from build123d import *

# Parameters (mm, degrees)
SKETCH1_W             = 70
SKETCH1_H             = 40
BOSS_EXTRUDE1_DEPTH   = 15
SKETCH2_W             = 60
SKETCH2_H             = 30
CUT_EXTRUDE1_DEPTH    = 51.249378106
CHAMFER1_SIZE         = 0.5
M4_TAPPED_HOLE1_D     = 3.3
M4_TAPPED_HOLE1_DEPTH = 11.5
M4_TAPPED_HOLE1_TIP   = 0.991420021
M4_TAPPED_HOLE2_D     = 3.3
CHAMFER3_SIZE         = 3
SKETCH17_W            = 10
SKETCH17_H            = 30
BOSS_EXTRUDE2_DEPTH   = 68.5
CHAMFER4_SIZE         = 0.5
M4_TAPPED_HOLE3_D     = 3.3
M4_TAPPED_HOLE3_DEPTH = 11.5
M4_TAPPED_HOLE3_TIP   = 0.991420021
CHAMFER5_SIZE         = 2
SKETCH20_R            = 2.5
CUT_EXTRUDE2_DEPTH    = 8
SKETCH21_W            = 3
SKETCH21_H            = 30
CUT_EXTRUDE3_DEPTH    = 114.829916981
CHAMFER6_SIZE         = 2


with BuildPart() as part:
    # Sketch1 → Boss-Extrude1 (new, symmetric)
    with BuildSketch(Plane.XY):
        Rectangle(SKETCH1_W, SKETCH1_H)
    extrude(amount=BOSS_EXTRUDE1_DEPTH, both=True)

    # Sketch2 → Cut-Extrude1 (cut, through all)
    with BuildSketch(Plane.XY.offset(15)):
        with Locations((-5, -5)):
            Rectangle(SKETCH2_W, SKETCH2_H)
    extrude(amount=-CUT_EXTRUDE1_DEPTH, mode=Mode.SUBTRACT)

    # Chamfer1
    chamfer1_edges = [part.edges().sort_by_distance(p)[0] for p in [
        (35, 0, 15),
        (35, 0, -15),
    ]]
    chamfer(chamfer1_edges, length=CHAMFER1_SIZE)

    # M4 Tapped Hole1
    with Locations(Plane(origin=(0, 20, 0), x_dir=(1, 0, 0), z_dir=(0, 1, 0))):
        with Locations((11, 0), (26, 0)):
            Hole(M4_TAPPED_HOLE1_D / 2, depth=M4_TAPPED_HOLE1_DEPTH)
            with Locations((0, 0, -(M4_TAPPED_HOLE1_DEPTH + M4_TAPPED_HOLE1_TIP / 2))):  # 118° drill point
                Cone(0, M4_TAPPED_HOLE1_D / 2, M4_TAPPED_HOLE1_TIP, mode=Mode.SUBTRACT)

    # M4 Tapped Hole2 (through all)
    with Locations(Plane(origin=(35, 0, 0), x_dir=(0, 0, -1), z_dir=(1, 0, 0))):
        with Locations((-10, 5), (-10, -15), (10, -15), (10, 5)):
            Hole(M4_TAPPED_HOLE2_D / 2)

    # Chamfer3
    chamfer3_edges = [part.edges().sort_by_distance(p)[0] for p in [
        (29.75, -20, -15),
        (29.75, -20, 15),
    ]]
    chamfer(chamfer3_edges, length=CHAMFER3_SIZE)

    # Sketch17 → Boss-Extrude2 (add)
    with BuildSketch(Plane(origin=(0, 20, 0), x_dir=(1, 0, 0), z_dir=(0, 1, 0))):
        with Locations((-30, 0)):
            Rectangle(SKETCH17_W, SKETCH17_H)
    extrude(amount=BOSS_EXTRUDE2_DEPTH)

    # Chamfer4
    chamfer4_edges = [part.edges().sort_by_distance(p)[0] for p in [
        (-25, 88.5, 0),
        (-35, 88.5, 0),
    ]]
    chamfer(chamfer4_edges, length=CHAMFER4_SIZE)

    # M4 Tapped Hole3
    with Locations(Plane(origin=(0, 88.5, 0), x_dir=(1, 0, 0), z_dir=(0, 1, 0))):
        with Locations((-30, 9), (-30, -9)):
            Hole(M4_TAPPED_HOLE3_D / 2, depth=M4_TAPPED_HOLE3_DEPTH)
            with Locations((0, 0, -(M4_TAPPED_HOLE3_DEPTH + M4_TAPPED_HOLE3_TIP / 2))):  # 118° drill point
                Cone(0, M4_TAPPED_HOLE3_D / 2, M4_TAPPED_HOLE3_TIP, mode=Mode.SUBTRACT)

    # Chamfer5
    chamfer5_edges = [part.edges().sort_by_distance(p)[0] for p in [
        (-35, 10, 0),
    ]]
    chamfer(chamfer5_edges, length=CHAMFER5_SIZE)

    # Sketch20 → Cut-Extrude2 (cut)
    with BuildSketch(Plane(origin=(0, 88.5, 0), x_dir=(1, 0, 0), z_dir=(0, 1, 0))):
        with Locations(Location((-30, 0, 0), (0, 0, 270))):
            Circle(SKETCH20_R)
    extrude(amount=-CUT_EXTRUDE2_DEPTH, mode=Mode.SUBTRACT)

    # Sketch21 → Cut-Extrude3 (cut, through all)
    with BuildSketch(Plane.ZY.offset(35)):
        with Locations((-13.5, 53.5)):
            Rectangle(SKETCH21_W, SKETCH21_H)
    cut_extrude3 = extrude(amount=-CUT_EXTRUDE3_DEPTH, mode=Mode.SUBTRACT)

    # Sketch22 → M4 Tapped Hole4 (revolve, cut)
    with BuildSketch(Plane(origin=(-30, 53.5, -12), x_dir=(0, 1, 0), z_dir=(1, 0, 0))):
        Polygon((0, 0), (0, 12.491420021), (1.65, 11.5), (1.65, 0), align=None)
    m4_tapped_hole4 = revolve(axis=Axis((-30, 53.5, -18.35), (0, 0, 1)), mode=Mode.SUBTRACT)

    # Mirror2: Cut-Extrude3, M4 Tapped Hole4 across plane
    add(cut_extrude3.mirror(Plane.XY), mode=Mode.SUBTRACT)
    add(m4_tapped_hole4.mirror(Plane.XY), mode=Mode.SUBTRACT)

    # Chamfer6
    chamfer6_edges = [part.edges().sort_by_distance(p)[0] for p in [
        (-30, 38.5, -15),
        (-30, 68.5, -15),
        (-30, 68.5, 15),
        (-30, 38.5, 15),
    ]]
    chamfer(chamfer6_edges, length=CHAMFER6_SIZE)


solid = part.part
For this review, take the finished solid that the model builds, in its own axes (mm). A direction names the side the tool comes from. Coordinates: 2 decimals unless noted, no trailing zeros. Loops run counter-clockwise (first coordinate to the right, second up) from the corner with the lowest first, then second, coordinate; pieces in that order, holes last. Notation, with made-up numbers: (52, 64) - (61, 64) arc R35 ccw to (61, 99) - close; hole circle Ø7 at (-8, -34.75). An arc over 180 degrees is marked (long way). Use a Markdown table: item, result. Add a question column.
Item 1: We need section B-B (y = 79). Give the boundary of the cut face in (x, z), and give its area (3 significant figures).
Item 2: We need section D-D (y = 58). Give the boundary of the cut face in (x, z).
Item 3: Mouldability with a two-part tool opening along Z and no side actions: class faces 1 (the face through (-30, 79, 15)), 2 (the face through (29.93, 3.536, 10.761)), 3 (the face through (-31.115, 52.284, 6.33)) as pulls with the +Z half, pulls with the -Z half, needs draft (parallel to the pull), parting line crosses it, or undercut.
Item 4: We need section A-A (y = -15). Give the boundary of the cut face in (x, z).
Item 5: Tool access review of faces 4 (the face through (-30, 80.5, 0)), 5 (the face through (25, -5, 0)), 6 (the face through (-30.1, 69.5, 14)), 7 (the face through (-25, 54, 0)): name each direction out of +Z, -Z, +X, -X, +Y, -Y from which nothing blocks a thin tool from reaching the whole face with its end or side.
Item 6: Insertion check: pin 1 Ø1.5 at (x, z) = (-30.5, 0.5) entering from +Y; pin 2 Ø4 at (x, z) = (6, 10.5) entering from -Y; pin 3 Ø1.5 at (y, z) = (43.5, -5.5) entering from +X; pin 4 Ø2.5 at (y, z) = (5, 10) entering from -X. Each pin has a flat end and moves straight along its axis. Give the tip position at first contact, or say it passes through.
Item 7: For line 1 (Y direction, x = 32.75, z = 10); line 2 (Y direction, x = -30, z = 9); line 3 (Y direction, x = 32.5, z = 6), list the stretches that pass through material, from the lowest coordinate up.
Item 8: We need section C-C (x = -4). Give the boundary of the cut face in (y, z), and give its area (3 significant figures).
Results list:
| question | item | result |
|---|---|---|
| 1 | outline | (-35, -15) - (-25, -15) - (-25, 15) - (-35, 15) - close; hole circle Ø3.3 at (-30, -9); hole circle Ø3.3 at (-30, 9) |
| 1 | area | 283 mm^2 |
| 2 | outline | (-35, -12) - (-25, -12) - (-25, 12) - (-35, 12) - close |
| 3 | face 1 | pulls with the +Z half |
| 3 | face 2 | undercut |
| 3 | face 3 | needs draft |
| 4 | outline | (25, -15) - (34.5, -15) - (35, -14.5) - (35, -11.65) - (25, -11.65) - close; (25, -8.35) - (35, -8.35) - (35, 8.35) - (25, 8.35) - close; (25, 11.65) - (35, 11.65) - (35, 14.5) - (34.5, 15) - (25, 15) - close |
| 5 | face 4 | +Y |
| 5 | face 5 | +Z, -Z, -X, -Y |
| 5 | face 6 | +Z, +X, -X |
| 5 | face 7 | +Z, -Z, +X, +Y |
| 6 | pin 1 | stops at y = 80.5 |
| 6 | pin 2 | stops at y = 10 |
| 6 | pin 3 | stops at x = -25 |
| 6 | pin 4 | passes through |
| 7 | line 1 | y = -20 to -16.65, -13.35 to 3.35, 6.65 to 20 |
| 7 | line 2 | y = 10 to 51.85, 55.15 to 76.01 |
| 7 | line 3 | y = -20 to 20 |
| 8 | outline | (10, -15) - (20, -15) - (20, 15) - (10, 15) - close |
| 8 | area | 300 mm^2 |
